Geometry check sheet. Reference: the model listing, model coordinates, mm. Face numbers are marked on the shaded views. A direction names the side the tool comes from. Give positions to 0.01 mm unless a question says otherwise; leave off trailing zeros. Loops run counter-clockwise (first coordinate to the right, second up) from the corner with the lowest first, then second, coordinate; pieces in that order, holes last. Notation, with made-up numbers: (81, 55) -> (117, 55) arc R19 ccw to (117, 87) -> close; hole circle Ø2 at (26, -36). An arc over 180 degrees is marked (long way). One line per item, written item: value. Start each with the question number.
(1) Sectioned sample at D-D, the plane x = 9. Record the cut outline in (y, z), then the cut area to 3 significant figures.
(2) Draft check along Y on the marked faces 1, 2 and 3. Enter one of: pulls with the +Y half, pulls with the -Y half, needs draft (parallel to the pull), parting line crosses it, or undercut.
(3) Gauge pin test, flat ends, axial feed: pin 1 Ø1 at (x, y) = (-1.5, 0.5) entering from +Z; pin 2 Ø1.1 at (x, y) = (12, 0) entering from +Z. Record the tip position at first contact, or that the pin passes through.
(4) Sectioned sample at B-B, the plane x = -2. Record the cut outline in (y, z).
(5) Scan lines: line 1 along Y through (x, z) = (12, -0.2) (3 decimals); line 2 along X through (y, z) = (-0.15, -0.35); line 3 along Y through (x, z) = (-5, -0.1). Record each from-to range of solid material in increasing order. Write a range as from..to.
(6) Tool access check on the marked faces 4, 5, 6, 7 and 8. Record the directions out of +Z, -Z, +X, -X, +Y, -Y that give a thin tool (end or side, any length) a straight path to the whole face; none if there is none.
(7) Sectioned sample at A-A, the plane y = 0. Record the cut outline in (x, z) (3 decimals).
(8) Sectioned sample at C-C, the plane z = 0.15. Record the cut outline in (x, y) (3 decimals), then the cut area to 3 significant figures.
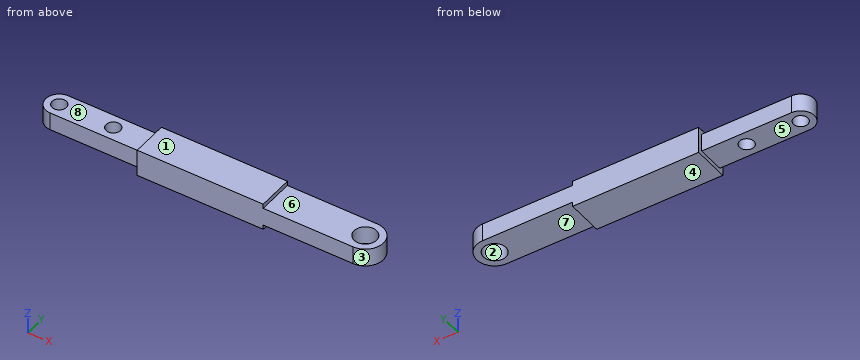
from build123d import *

# Parameters (mm, degrees)
SKETCH1_R           = 0.625
BOSS_EXTRUDE1_DEPTH = 0.75
SKETCH3_R           = 0.4
BOSS_EXTRUDE3_DEPTH = 0.5
CUT_EXTRUDE1_START  = -0.25
CUT_EXTRUDE1_DEPTH  = 0.25


with BuildPart() as part:
    # Sketch1 → Boss-Extrude1 (new, symmetric)
    with BuildSketch(Plane.XY):
        with BuildLine():
            Line((0, -1), (0, 1))
            Line((0, 1), (12, 1))
            ThreePointArc((12, 1), (13, 0), (12, -1))
            Line((12, -1), (0, -1))
        make_face()
        with Locations((12, 0)):
            Circle(SKETCH1_R, mode=Mode.SUBTRACT)
    extrude(amount=BOSS_EXTRUDE1_DEPTH, both=True)

    # Sketch3 → Boss-Extrude3 (add, symmetric)
    with BuildSketch(Plane.XY):
        with BuildLine():
            Line((0, -0.75), (-5, -0.75))
            ThreePointArc((-5, -0.75), (-5.75, 0), (-5, 0.75))
            Line((-5, 0.75), (0, 0.75))
            Line((0, 0.75), (0, -0.75))
        make_face()
        with Locations((-5, 0)):
            Circle(SKETCH3_R, mode=Mode.SUBTRACT)
        with Locations((-2, 0)):
            Circle(SKETCH3_R, mode=Mode.SUBTRACT)
    extrude(amount=BOSS_EXTRUDE3_DEPTH, both=True)

    # Sketch6 → Cut-Extrude1 (cut)
    with BuildSketch(Plane(origin=(0, 0, -0.75), x_dir=(-1, 0, 0), z_dir=(0, 0, -1)).offset(CUT_EXTRUDE1_START)):
        with BuildLine():
            Line((-7, 1), (-7, -1))
            Line((-7, -1), (-12, -1))
            ThreePointArc((-12, -1), (-13, 0), (-12, 1))
            Line((-12, 1), (-7, 1))
        make_face()
    cut_extrude1 = extrude(amount=CUT_EXTRUDE1_DEPTH, mode=Mode.SUBTRACT)

    # Mirror1: Cut-Extrude1 across plane
    add(cut_extrude1.mirror(Plane.XY), mode=Mode.SUBTRACT)


solid = part.part
Calculated:
1. outline: (-1, -0.5) -> (1, -0.5) -> (1, 0.5) -> (-1, 0.5) -> close
1. area: 2.00 mm2
2. face 1: needs draft
2. face 2: undercut
2. face 3: parting line crosses it
3. pin 1: stops at z = 0.5
3. pin 2: passes through
4. outline: (-0.75, -0.5) -> (-0.4, -0.5) -> (-0.4, 0.5) -> (-0.75, 0.5) -> close; (0.4, -0.5) -> (0.75, -0.5) -> (0.75, 0.5) -> (0.4, 0.5) -> close
5. line 1: y = -1..-0.625, 0.625..1
5. line 2: x = -5.73..-5.37, -4.63..-2.37, -1.63..11.39, 12.61..12.99
5. line 3: y = -0.75..-0.4, 0.4..0.75
6. face 4: -Z, +X, -X, +Y, -Y
6. face 5: -Z, -X, +Y, -Y
6. face 6: +Z, +X, +Y, -Y
6. face 7: -Z, +X, +Y, -Y
6. face 8: +Z, -X, +Y, -Y
7. outline: (-5.75, -0.5) -> (-5.4, -0.5) -> (-5.4, 0.5) -> (-5.75, 0.5) -> close; (-4.6, -0.5) -> (-2.4, -0.5) -> (-2.4, 0.5) -> (-4.6, 0.5) -> close; (-1.6, -0.5) -> (0, -0.5) -> (0, -0.75) -> (7, -0.75) -> (7, -0.5) -> (11.375, -0.5) -> (11.375, 0.5) -> (7, 0.5) -> (7, 0.75) -> (0, 0.75) -> (0, 0.5) -> (-1.6, 0.5) -> close; (12.625, -0.5) -> (13, -0.5) -> (13, 0.5) -> (12.625, 0.5) -> close
8. outline: (-5, -0.75) -> (0, -0.75) -> (0, -1) -> (12, -1) arc R1 ccw to (12, 1) -> (0, 1) -> (0, 0.75) -> (-5, 0.75) arc R0.75 ccw to start; hole circle Ø0.8 at (-5, 0); hole circle Ø0.8 at (-2, 0); hole circle Ø1.25 at (12, 0)
8. area: 31.7 mm2
